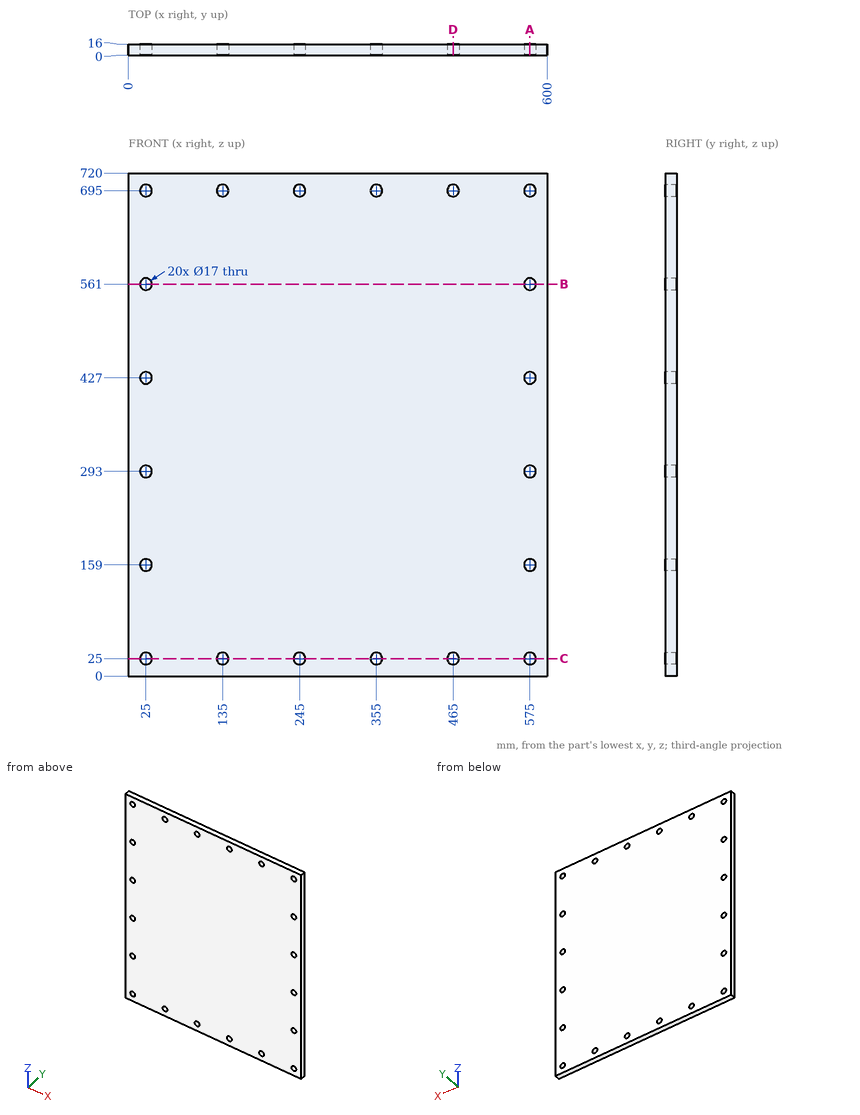
Source: three-view drawing plus pictorial views. Frame: mm from the lowest corner of the part. Round coordinates to 2 decimals unless told otherwise and drop trailing zeros. Loops run counter-clockwise (first coordinate to the right, second up) from the corner with the lowest first, then second, coordinate; pieces in that order, holes last.
1. Section query A-A on x = 575. Output: boundary loops of the cut face in (y, z).
2. Ray query, L1, parallel to X at y = 10.75, z = 293; L2, parallel to Z at x = 252.5, y = 13; L3, parallel to Z at x = 250.5, y = 13. Return the intervals inside material, ascending.
3. Section query C-C on z = 25. Output: boundary loops of the cut face in (x, y).
4. Section query B-B on z = 561. Output: boundary loops of the cut face in (x, y), and give its area (3 significant figures).
5. Section query D-D on x = 465. Output: boundary loops of the cut face in (y, z), and give its area (3 significant figures).
6. Contact query for a flat-ended pin moving along its axis: pin 1 (13.5 mm diameter, centred on x = 25, z = 561, fed in from -Y). Output: stop coordinate, or through.
Answers below:
1. outline: (0, 0) - (16, 0) - (16, 16.5) - (0, 16.5) - close; (0, 33.5) - (16, 33.5) - (16, 150.5) - (0, 150.5) - close; (0, 167.5) - (16, 167.5) - (16, 284.5) - (0, 284.5) - close; (0, 301.5) - (16, 301.5) - (16, 418.5) - (0, 418.5) - close; (0, 435.5) - (16, 435.5) - (16, 552.5) - (0, 552.5) - close; (0, 569.5) - (16, 569.5) - (16, 686.5) - (0, 686.5) - close; (0, 703.5) - (16, 703.5) - (16, 720) - (0, 720) - close
2. L1: x = 0 to 16.5, 33.5 to 566.5, 583.5 to 600
2. L2: z = 0 to 21, 29 to 691, 699 to 720
2. L3: z = 0 to 18.52, 31.48 to 688.52, 701.48 to 720
3. outline: (0, 0) - (16.5, 0) - (16.5, 16) - (0, 16) - close; (33.5, 0) - (126.5, 0) - (126.5, 16) - (33.5, 16) - close; (143.5, 0) - (236.5, 0) - (236.5, 16) - (143.5, 16) - close; (253.5, 0) - (346.5, 0) - (346.5, 16) - (253.5, 16) - close; (363.5, 0) - (456.5, 0) - (456.5, 16) - (363.5, 16) - close; (473.5, 0) - (566.5, 0) - (566.5, 16) - (473.5, 16) - close; (583.5, 0) - (600, 0) - (600, 16) - (583.5, 16) - close
4. outline: (0, 0) - (16.5, 0) - (16.5, 16) - (0, 16) - close; (33.5, 0) - (566.5, 0) - (566.5, 16) - (33.5, 16) - close; (583.5, 0) - (600, 0) - (600, 16) - (583.5, 16) - close
4. area: 9,060 mm2
5. outline: (0, 0) - (16, 0) - (16, 16.5) - (0, 16.5) - close; (0, 33.5) - (16, 33.5) - (16, 686.5) - (0, 686.5) - close; (0, 703.5) - (16, 703.5) - (16, 720) - (0, 720) - close
5. area: 11,000 mm2
6. pin 1: passes through
